Here's how the part is built. I have some questions about the finished solid (model axes, mm). A direction names the side the tool comes from. Round coordinates to 2 decimals unless told otherwise and drop trailing zeros. Loops run counter-clockwise (first coordinate to the right, second up) from the corner with the lowest first, then second, coordinate; pieces in that order, holes last. Notation, with made-up numbers: M 87,24.25 L 132,24.25 A32 ccw 132,62.25 Z; hole C 38.5,58.5 d1. An arc over 180 degrees is marked long. Use a Markdown table: item, result.
from build123d import *

# Parameters (mm, degrees)
BOSS_EXTRUDE1_DEPTH = 2240
SHELL1_T            = -4


with BuildPart() as part:
    # Sketch1 → Boss-Extrude1 (new body)
    with BuildSketch(Plane.XY):
        with BuildLine():
            Line((55, 25), (-55, 25))
            ThreePointArc((-55, 25), (-58.535533906, 23.535533906), (-60, 20))
            Line((-60, 20), (-60, -20))
            ThreePointArc((-60, -20), (-58.535533906, -23.535533906), (-55, -25))
            Line((-55, -25), (55, -25))
            ThreePointArc((55, -25), (58.535533906, -23.535533906), (60, -20))
            Line((60, -20), (60, 20))
            ThreePointArc((60, 20), (58.535533906, 23.535533906), (55, 25))
        make_face()
    extrude(amount=BOSS_EXTRUDE1_DEPTH)

    # Shell1
    shell1_openings = [part.faces().sort_by_distance(p)[0] for p in [
        (0, 0, 2240),
        (0, 0, 0),
    ]]
    offset(amount=SHELL1_T, openings=shell1_openings, kind=Kind.INTERSECTION)


solid = part.part
1. We'd pull the mould along Y, two halves only. Please class faces 1 (the face through (1, 25, 1104)), 2 (the face through (-1, -25, 1104)), 3 (the face through (1, 21, 1104)): +Y half, -Y half, draft (parallel to the pull), parting line (faces both ways), or undercut.
Answer sheet:
| item | result |
|---|---|
| face 1 | +Y half |
| face 2 | -Y half |
| face 3 | undercut |
2. Which directions (+Z, -Z, +X, -X, +Y, -Y) give clear straight access to the entire face, cutting with the end or side of a thin tool? Please do faces 4 (the face through (-56, 0, 1104)), 5 (the face through (0, -22, 2240)).
Answer sheet:
| item | result |
|---|---|
| face 4 | +Z, -Z |
| face 5 | +Z, +X, -X, +Y, -Y |
3. Imagine slicing it at B-B, the plane x = -36. Write out the boundary of the cut face in (y, z), then the cut area to 3 significant figures.
Answer sheet:
| item | result |
|---|---|
| outline | M -25,0 L -21,0 L -21,2240 L -25,2240 Z; M 21,0 L 25,0 L 25,2240 L 21,2240 Z |
| area | 17,900 mm2 |
4. Imagine slicing it at C-C, the plane z = 198. Write out the boundary of the cut face in (x, y).
Answer sheet:
| item | result |
|---|---|
| outline | M -60,-20 A5 ccw -55,-25 L 55,-25 A5 ccw 60,-20 L 60,20 A5 ccw 55,25 L -55,25 A5 ccw -60,20 Z; hole M -56,-20 A1 ccw -55,-21 L 55,-21 A1 ccw 56,-20 L 56,20 A1 ccw 55,21 L -55,21 A1 ccw -56,20 Z |
5. I need wall thicknesses on probe 1 along X at (y, z) = (14, 1326.5); probe 2 along Y at (x, z) = (45, 144.5); probe 3 along X at (y, z) = (-20.5, 948.5). Which ranges of each line are inside material? Lowest first, please. Write a range as from..to.
Answer sheet:
| item | result |
|---|---|
| probe 1 | -60..-56, 56..60 |
| probe 2 | -25..-21, 21..25 |
| probe 3 | -59.97..-55.87, 55.87..59.97 |
6. Imagine slicing it at A-A, the plane y = 0. Write out the boundary of the cut face in (x, z), then the cut area to 3 significant figures.
Answer sheet:
| item | result |
|---|---|
| outline | M -60,0 L -56,0 L -56,2240 L -60,2240 Z; M 56,0 L 60,0 L 60,2240 L 56,2240 Z |
| area | 17,900 mm2 |
